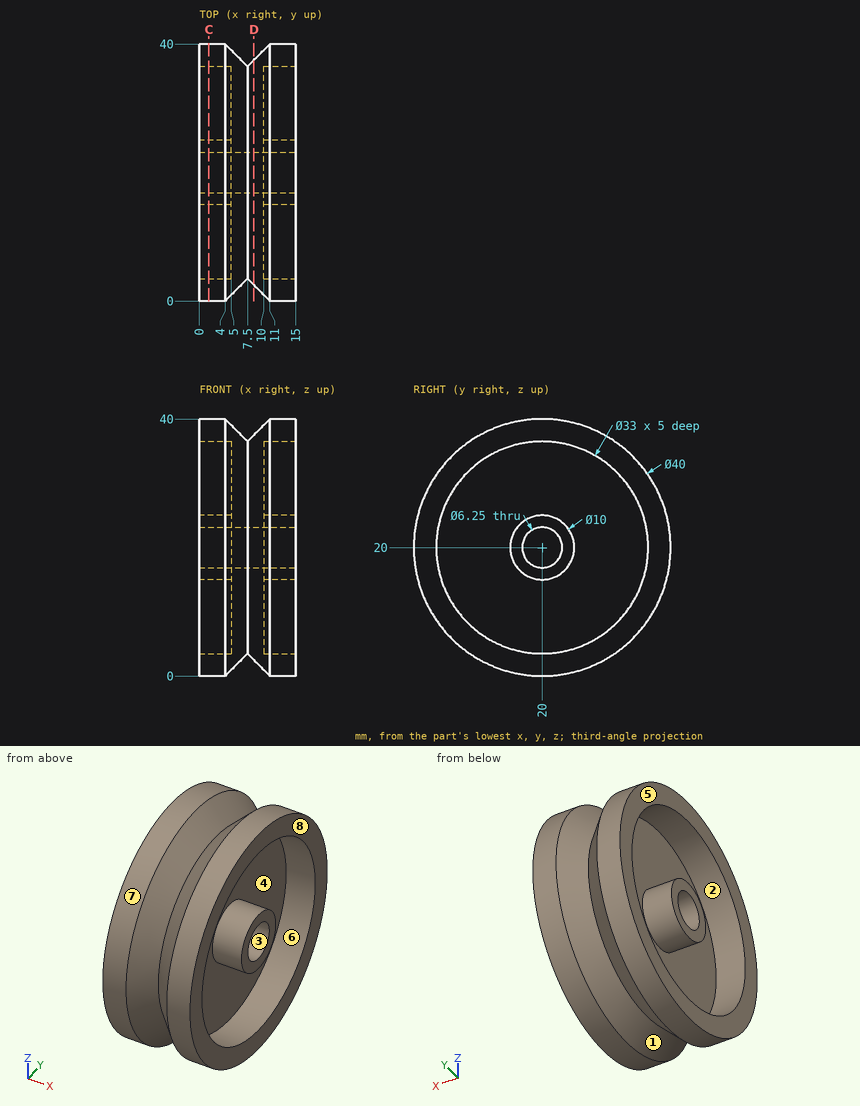
Can you work these out from the drawing? Everything is in mm from the part's minimum corner. A direction names the side the tool comes from. Coordinates: 2 decimals unless noted, no trailing zeros. Loops run counter-clockwise (first coordinate to the right, second up) from the corner with the lowest first, then second, coordinate; pieces in that order, holes last. Notation, with made-up numbers: (-30.75, 0.25) - (15.25, 0.25) arc R16 cw to (15.25, 6.25) - close; hole circle Ø3 at (39.5, -8.75). An arc over 180 degrees is marked (long way). Answer as CSV lines item,"result".
Q1. For pin 1 (5 mm diameter, centred on x = 5, y = 35, fed in from +Z); pin 2 (4 mm diameter, centred on x = 8, z = 8, fed in from +Y); pin 3 (6 mm diameter, centred on x = 3.5, y = 35, fed in from -Z), each with a flat end and sliding along its axis, tell me the tip position at first contact or that it passes through.
Response:
pin 1,"z = 35.44"
pin 2,"y = 35.16"
pin 3,"z = 4"
Q2. For the marked faces 1, 2, 3, 4 and 5, which set-ups out of +Z, -Z, +X, -X, +Y, -Y let a thin tool reach every point of the face, with its end or its side?
Response:
face 1,"none"
face 2,"-X"
face 3,"+X, -X"
face 4,"+X"
face 5,"+Z, -Z, -X, +Y, -Y"
Q3. If we section it at C-C, the plane x = 1.5: Write out the boundary of the cut face in (y, z) (3 decimals), and give its area (3 significant figures).
Response:
outline,"circle Ø40 at (20, 20); circle Ø10 at (20, 20); hole circle Ø33 at (20, 20); hole circle Ø6.25 at (20, 20)"
area,"449 mm2"
Q4. If we section it at D-D, the plane x = 8.5: Write out the boundary of the cut face in (y, z) (3 decimals).
Response:
outline,"circle Ø35 at (20, 20); hole circle Ø6.25 at (20, 20)"
Q5. If I drill on L1, parallel to Y at x = 2.5, z = 20 (3 decimals); L2, parallel to Y at x = 10.75, z = 20.5; L3, parallel to X at y = 27.5, z = 26, over which ranges is the centre line in solid material (lowest first)? Write a range as [from, to].
Response:
L1,"[0, 3.5], [15, 16.875], [23.125, 25], [36.5, 40]"
L2,"[0.26, 3.51], [15.03, 16.92], [23.08, 24.97], [36.49, 39.74]"
L3,"[5, 10]"
Q6. We'd pull the mould along Y, two halves only. Please class the marked faces 6, 7 and 8: pulls with the +Y half, pulls with the -Y half, needs draft (parallel to the pull), parting line crosses it, or undercut.
Response:
face 6,"undercut"
face 7,"parting line crosses it"
face 8,"needs draft"
